from build123d import *

# Parameters (mm, degrees)
SKETCH_1_W                  = 30
SKETCH_1_H                  = 30
EXTRUDE_1_DEPTH             = 5
SKETCH_2_W                  = 30
SKETCH_2_H                  = 5
EXTRUDE_2_DEPTH             = 17
HOLE_WIZARD_3_5_3_5_1_D     = 3.5
HOLE_WIZARD_3_5_3_5_1_DEPTH = 12.4
HOLE_WIZARD_3_5_3_5_1_TIP   = 1.051506083
SKETCH_5_W                  = 20.75
SKETCH_5_H                  = 1
CUT_EXTRUDE_1_DEPTH         = 41.11234224
CHAMFER_1_SIZE              = 2
HOLE_WIZARD_3_5_3_5_2_D     = 3.5
HOLE_WIZARD_3_5_3_5_2_DEPTH = 12.4
HOLE_WIZARD_3_5_3_5_2_TIP   = 1.051506083
MM_1_D                      = 3
MM_1_DEPTH                  = 12.4
MM_1_TIP                    = 0.901290929


with BuildPart() as part:
    # 草图1 → 凸台-拉伸1 (new body)
    with BuildSketch(Plane(origin=(0, 0, 0), x_dir=(1, 0, 0), z_dir=(0, 1, 0))):
        Rectangle(SKETCH_1_W, SKETCH_1_H)
    extrude(amount=EXTRUDE_1_DEPTH)

    # 草图2 → 凸台-拉伸2 (add)
    with BuildSketch(Plane(origin=(0, 5, 0), x_dir=(1, 0, 0), z_dir=(0, 1, 0))):
        with Locations((0, -12.5)):
            Rectangle(SKETCH_2_W, SKETCH_2_H)
    extrude(amount=EXTRUDE_2_DEPTH)

    # Ø3.5 (3.5) 直径孔1
    with Locations(Plane(origin=(0, 5, 0), x_dir=(1, 0, 0), z_dir=(0, 1, 0))):
        with Locations((-5, 11.75), (5, 11.75), (5, -3.25), (-5, -3.25)):
            Hole(HOLE_WIZARD_3_5_3_5_1_D / 2, depth=HOLE_WIZARD_3_5_3_5_1_DEPTH)
            with Locations((0, 0, -(HOLE_WIZARD_3_5_3_5_1_DEPTH + HOLE_WIZARD_3_5_3_5_1_TIP / 2))):  # 118° drill point
                Cone(0, HOLE_WIZARD_3_5_3_5_1_D / 2, HOLE_WIZARD_3_5_3_5_1_TIP, mode=Mode.SUBTRACT)

    # 草图5 → 切除-拉伸1 (cut, through all)
    with BuildSketch(Plane.ZY.offset(15)):
        with Locations((-4.625, 0.5)):
            Rectangle(SKETCH_5_W, SKETCH_5_H)
    extrude(amount=-CUT_EXTRUDE_1_DEPTH, mode=Mode.SUBTRACT)

    # 倒角1
    chamfer_1_edges = [part.edges().sort_by_distance(p)[0] for p in [
        (-15, 22, 12.5),
        (15, 22, 12.5),
        (-15, 3, -15),
        (15, 3, -15),
    ]]
    chamfer(chamfer_1_edges, length=CHAMFER_1_SIZE)

    # Ø3.5 (3.5) 直径孔2
    with Locations(Plane(origin=(0, 0, 10), x_dir=(-1, 0, 0), z_dir=(0, 0, -1))):
        with Locations((-10, 17), (10, 17), (-10, 9), (10, 9)):
            Hole(HOLE_WIZARD_3_5_3_5_2_D / 2, depth=HOLE_WIZARD_3_5_3_5_2_DEPTH)
            with Locations((0, 0, -(HOLE_WIZARD_3_5_3_5_2_DEPTH + HOLE_WIZARD_3_5_3_5_2_TIP / 2))):  # 118° drill point
                Cone(0, HOLE_WIZARD_3_5_3_5_2_D / 2, HOLE_WIZARD_3_5_3_5_2_TIP, mode=Mode.SUBTRACT)

    # 大小mm 暗销孔1
    with Locations(Plane(origin=(0, 0, 10), x_dir=(-1, 0, 0), z_dir=(0, 0, -1))):
        with Locations((0, 17), (0, 9)):
            Hole(MM_1_D / 2, depth=MM_1_DEPTH)
            with Locations((0, 0, -(MM_1_DEPTH + MM_1_TIP / 2))):  # 118° drill point
                Cone(0, MM_1_D / 2, MM_1_TIP, mode=Mode.SUBTRACT)


solid = part.part
Geometry: final body of the model. Coordinates: model frame, mm. A direction names the side the tool comes from. Round coordinates to 2 decimals unless told otherwise and drop trailing zeros. Loops run counter-clockwise (first coordinate to the right, second up) from the corner with the lowest first, then second, coordinate; pieces in that order, holes last. Notation, with made-up numbers: M -17.5,74 L 23.5,74 A17 ccw 23.5,94 Z; hole C 86.5,68.25 d8. An arc over 180 degrees is marked long. Put each result on its own line as item: value. Start each with the question number.
(1) Contact query for flat-ended pins moving along their axis: pin 1 Ø4.5 at (x, z) = (5, 3.25) entering from +Y; pin 2 Ø4 at (x, y) = (10, 9) entering from -Z; pin 3 Ø10.5 at (x, z) = (1.5, -3) entering from -Y. Output: stop coordinate, or through.
(2) Draft query along X for faces 3 (the face through (0, 13, 10)), 4 (the face through (14, 21, 13)), 5 (the face through (10.9, 10.5, 12.5)). Return one class per face: +X half, -X half, draft (parallel to the pull), parting line (faces both ways), or undercut.
(3) Section query B-B (y = 9). Return loops of the section in (x, z).
(4) Material intervals for line 1 along Y through (x, z) = (-10, 12.3); line 2 along Z through (x, y) = (5, 1.95); line 3 along X through (y, z) = (3.5, -11.75), sorted ascending. Write a range as [from, to].
(5) Section query D-D (x = -10). Return loops of the section in (y, z), then the cut area to 3 significant figures.
(6) Section query C-C (z = -11.75). Return loops of the section in (x, y), then the cut area to 3 significant figures.
(7) Set-up query: faces 1 (the face through (15, 4.8, 5.2)), 2 (the face through (-0.2, 0.5, 5.75)). Return all of +Z, -Z, +X, -X, +Y, -Y with unobstructed straight access to the full face (end or side cutting, diameter ignored); none if empty.
(8) Section query A-A (x = 5). Return loops of the section in (y, z).
Findings below:
1. pin 1: stops at y = 5
1. pin 2: stops at z = 10
1. pin 3: stops at y = 1
2. face 3: draft
2. face 4: +X half
2. face 5: undercut
3. outline: M -15,10 L -11.75,10 L -11.75,15 L -15,15 Z; M -8.25,10 L -1.5,10 L -1.5,15 L -8.25,15 Z; M 1.5,10 L 8.25,10 L 8.25,15 L 1.5,15 Z; M 11.75,10 L 15,10 L 15,15 L 11.75,15 Z
4. line 1: y = [0, 7.25], [10.75, 15.25], [18.75, 22]
4. line 2: z = [-15, -13.5], [-10, 1.5], [5, 15]
4. line 3: x = [-15, -6.75], [-3.25, 3.25], [6.75, 15]
5. outline: M 0,5.75 L 1,5.75 L 1,-15 L 5,-15 L 5,10 L 7.25,10 L 7.25,15 L 0,15 Z; M 10.75,10 L 15.25,10 L 15.25,15 L 10.75,15 Z; M 18.75,10 L 22,10 L 22,15 L 18.75,15 Z
5. area: 179 mm2
6. outline: M -15,1 L -6.75,1 L -6.75,5 L -15,5 Z; M -3.25,1 L 3.25,1 L 3.25,5 L -3.25,5 Z; M 6.75,1 L 15,1 L 15,5 L 6.75,5 Z
6. area: 92.0 mm2
7. face 1: +Z, -Z, +X, +Y, -Y
7. face 2: -Z, +X, -X, -Y
8. outline: M 0,5.75 L 1,5.75 L 1,5 L 5,5 L 5,10 L 22,10 L 22,15 L 0,15 Z; M 1,-15 L 5,-15 L 5,-13.5 L 1,-13.5 Z; M 1,-10 L 5,-10 L 5,1.5 L 1,1.5 Z
